Answer from the drawing. Dimensions are ordinates in mm from the lowest x, y and z of the part. Give positions to 0.01 mm unless a question says otherwise; leave off trailing zeros. Loops run counter-clockwise (first coordinate to the right, second up) from the corner with the lowest first, then second, coordinate; pieces in that order, holes last. Notation, with made-up numbers: (42, 10.5) - (52, 10.5) arc R24 ccw to (52, 45.5) - close; hole circle Ø1 at (-34.75, -13). An arc over 180 degrees is marked (long way). One line per item, written item: value.
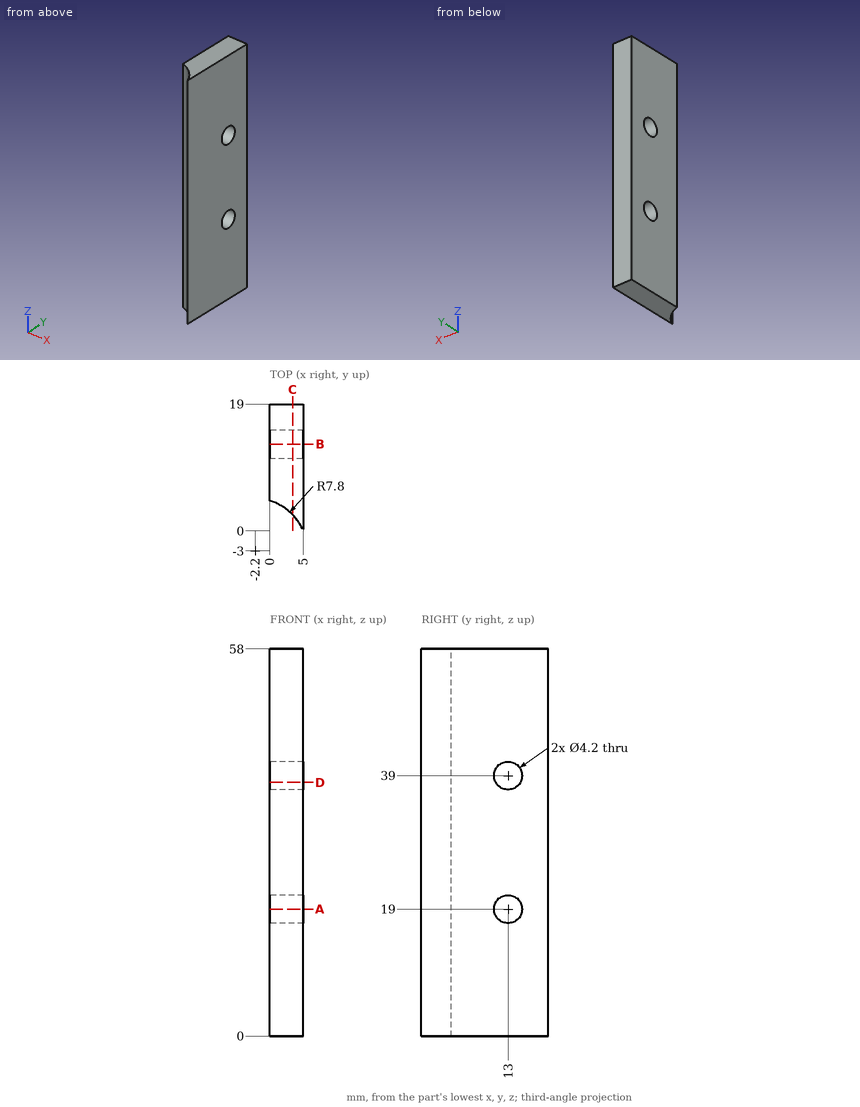
1. Section A-A (z = 19) is taken. Write down the section's boundary in (x, y).
Output:
outline: (0, 4.48) arc R7.8 cw to (5, 0) - (5, 10.9) - (0, 10.9) - close; (0, 15.1) - (5, 15.1) - (5, 19) - (0, 19) - close
2. Section B-B (y = 13) is taken. Write down the section's boundary in (x, z).
Output:
outline: (0, 0) - (5, 0) - (5, 16.9) - (0, 16.9) - close; (0, 21.1) - (5, 21.1) - (5, 36.9) - (0, 36.9) - close; (0, 41.1) - (5, 41.1) - (5, 58) - (0, 58) - close
3. Find the intervals of material crossed by line 1 along Z through (x, y) = (2.1, 13); line 2 along Y through (x, z) = (1.85, 21.5); line 3 along Y through (x, z) = (2.1, 10), in increasing order.
Output:
line 1: z = 0 to 16.9, 21.1 to 36.9, 41.1 to 58
line 2: y = 3.67 to 19
line 3: y = 3.51 to 19
4. A flat-ended cylindrical pin translates along its axis: pin 1 Ø3 at (x, z) = (2.5, 35.5) entering from -Y. Find the tip coordinate at first contact, or state that the pin passes through.
Output:
pin 1: stops at y = 1.73
5. Section D-D (z = 38) is taken. Write down the section's boundary in (x, y).
Output:
outline: (0, 4.48) arc R7.8 cw to (5, 0) - (5, 11.15) - (0, 11.15) - close; (0, 14.85) - (5, 14.85) - (5, 19) - (0, 19) - close
6. Section C-C (x = 3.4) is taken. Write down the section's boundary in (y, z).
Output:
outline: (2.43, 0) - (19, 0) - (19, 58) - (2.43, 58) - close; hole circle Ø4.2 at (13, 19); hole circle Ø4.2 at (13, 39)
